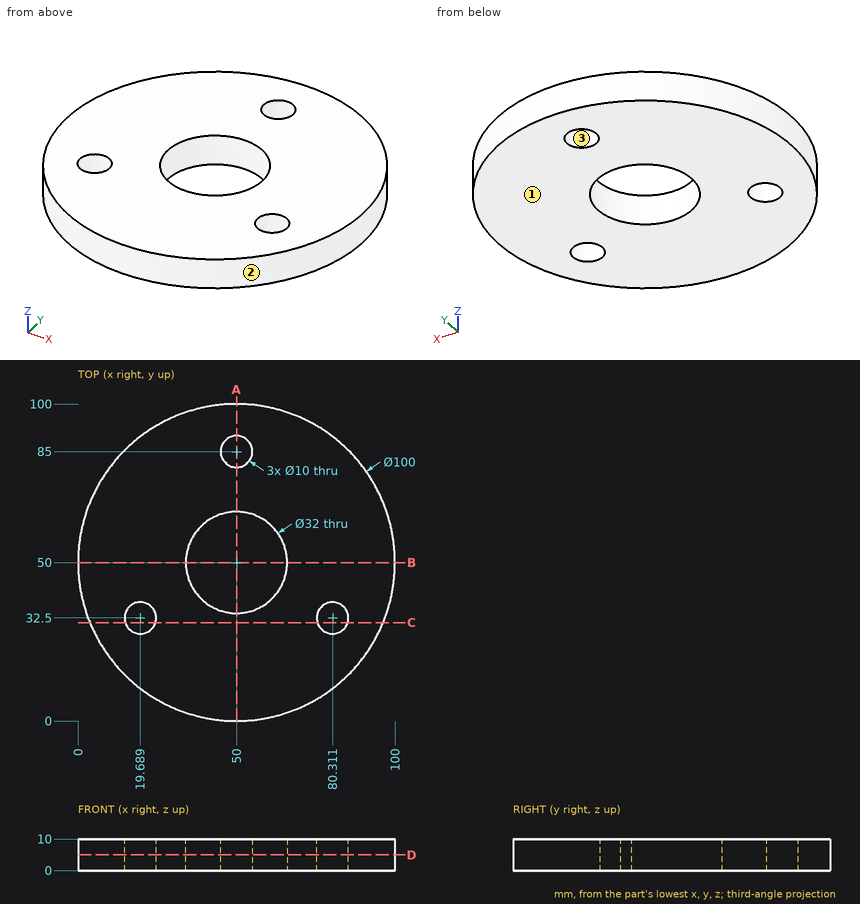
Could you check a few things on this drawing? It's one solid part, dimensions in mm from its lowest x, y, z. Coordinates: 2 decimals unless noted, no trailing zeros. Order: outer loops, then holes, each group sorted by start corner. A loop starts at its lowest first (then second) coordinate and runs counter-clockwise, first axis right, second up. Notation, with made-up numbers: (61, 15.25) - (107, 15.25) arc R10 cw to (107, 19.25) - close; hole circle Ø8 at (74.5, -17). An arc over 180 degrees is marked (long way). One line per question, with ' | ' between items. Start each with the question number.
1. Please list where these lines run through material, in increasing order: line 1 along Y through (x, z) = (50, 7.75); line 2 along X through (y, z) = (29, 5.25); line 3 along Y through (x, z) = (22, 5.5) (1 decimal). Write a range as [from, to].
2. If we section it at A-A (x = 50): Write out the boundary of the cut face in (y, z), and give its area (3 significant figures).
3. If we mould it in two halves opening along Y, with no side actions, what happens to the marked faces 1, 2 and 3? For each: released by +Y, released by -Y, zero draft, split by the parting line, or undercut.
4. I'm going to push flat-ended pins straight in: pin 1 Ø5 at (y, z) = (35, 6.5) entering from +X; pin 2 Ø6 at (x, z) = (15.5, 7) entering from -Y; pin 3 Ø5 at (x, z) = (72.5, 7) entering from +Y. Where does each tip first touch, or does it pass through?
5. If we section it at B-B (y = 50): Write out the boundary of the cut face in (x, z).
6. If we section it at C-C (y = 31): Write out the boundary of the cut face in (x, z).
7. If we section it at D-D (z = 5): Write out the boundary of the cut face in (x, y).
Model answer:
1) line 1: y = [0, 34], [66, 80], [90, 100] | line 2: x = [4.62, 16.12], [23.26, 76.74], [83.88, 95.38] | line 3: y = [8.6, 28.1], [36.9, 91.4]
2) outline: (0, 0) - (34, 0) - (34, 10) - (0, 10) - close; (66, 0) - (80, 0) - (80, 10) - (66, 10) - close; (90, 0) - (100, 0) - (100, 10) - (90, 10) - close | area: 580 mm²
3) face 1: zero draft | face 2: split by the parting line | face 3: undercut
4) pin 1: stops at x = 98.41 | pin 2: stops at y = 11.17 | pin 3: stops at y = 95.83
5) outline: (0, 0) - (34, 0) - (34, 10) - (0, 10) - close; (66, 0) - (100, 0) - (100, 10) - (66, 10) - close
6) outline: (3.75, 0) - (14.92, 0) - (14.92, 10) - (3.75, 10) - close; (24.46, 0) - (75.54, 0) - (75.54, 10) - (24.46, 10) - close; (85.08, 0) - (96.25, 0) - (96.25, 10) - (85.08, 10) - close
7) outline: circle Ø100 at (50, 50); hole circle Ø10 at (19.69, 32.5); hole circle Ø32 at (50, 50); hole circle Ø10 at (50, 85); hole circle Ø10 at (80.31, 32.5)
